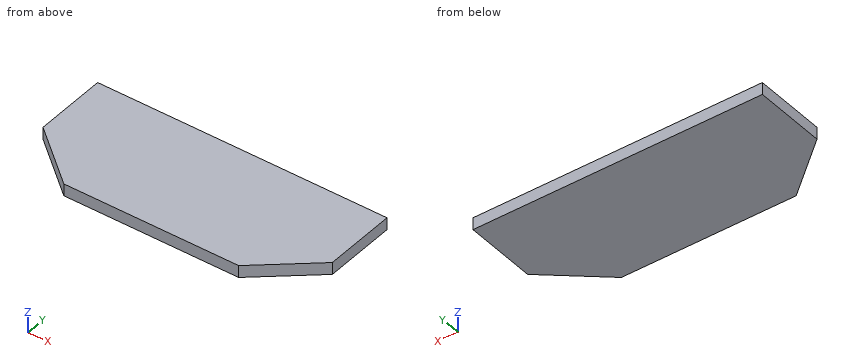
```python
from build123d import *

# Parameters (mm, degrees)
EXTRUDE_1_DEPTH = 10


with BuildPart() as part:
    # 草图1 → 凸台-拉伸1 (new body)
    with BuildSketch(Plane.XY):
        Polygon((120, 0), (-120, 0), (-120, -60), (-72.5, -100), (72.5, -100), (120, -60), align=None)
    extrude(amount=EXTRUDE_1_DEPTH)


solid = part.part
```
Source: CAD feature listing. Evaluate the final solid. Frame: model axes, mm. Round coordinates to 2 decimals unless told otherwise and drop trailing zeros. Loops run counter-clockwise (first coordinate to the right, second up) from the corner with the lowest first, then second, coordinate; pieces in that order, holes last. Notation, with made-up numbers: (-40, 76.5) - (-8, 76.5) arc R22 ccw to (-8, 112.5) - close; hole circle Ø8 at (1, -19.5). An arc over 180 degrees is marked (long way). Use CSV: the item, a comma, the result in double quotes.
Q1. Section query C-C, the plane y = -83.5. Output: boundary loops of the cut face in (x, z).
Reported:
outline,"(-92.09, 0) - (92.09, 0) - (92.09, 10) - (-92.09, 10) - close"
Q2. Ray query, line 1 along Y through (x, z) = (107, 4.75); line 2 along X through (y, z) = (-80.5, 3); line 3 along Y through (x, z) = (-105, 3). Return the intervals inside material, ascending.
Reported:
line 1,"-70.95 to 0"
line 2,"-95.66 to 95.66"
line 3,"-72.63 to 0"
Q3. Section query B-B, the plane x = -89. Output: boundary loops of the cut face in (y, z), then the cut area to 3 significant figures.
Reported:
outline,"(-86.11, 0) - (0, 0) - (0, 10) - (-86.11, 10) - close"
area,"861 mm^2"
Q4. Section query A-A, the plane z = 6.25. Output: boundary loops of the cut face in (x, y), then the cut area to 3 significant figures.
Reported:
outline,"(-120, -60) - (-72.5, -100) - (72.5, -100) - (120, -60) - (120, 0) - (-120, 0) - close"
area,"22,100 mm^2"
